Geometry: final body of the model. Coordinates: model frame, mm. Coordinates: 2 decimals unless noted, no trailing zeros. Write each loop counter-clockwise with the first axis right and the second up, starting at its lowest first coordinate (ties: lowest second). Pieces come first, ordered by that corner, then holes. Notation, with made-up numbers: (62.5, 40.25) -> (117.5, 40.25) arc R27 cw to (117.5, 76.25) -> close; hole circle Ø4 at (35, -24.5). An arc over 180 degrees is marked (long way). One line per item, written item: value.
```python
from build123d import *

# Parameters (mm, degrees)
SKETCH1_R           = 25
SKETCH1_R_2         = 9
SKETCH1_R_3         = 2.1
BOSS_EXTRUDE1_DEPTH = 4


with BuildPart() as part:
    # Sketch1 → Boss-Extrude1 (new body)
    with BuildSketch(Plane.XY):
        Circle(SKETCH1_R)
        Circle(SKETCH1_R_2, mode=Mode.SUBTRACT)
        with Locations((0, 20)):
            Circle(SKETCH1_R_3, mode=Mode.SUBTRACT)
        with Locations((-20, 0)):
            Circle(SKETCH1_R_3, mode=Mode.SUBTRACT)
        with Locations((20, 0)):
            Circle(SKETCH1_R_3, mode=Mode.SUBTRACT)
        with Locations((0, -20)):
            Circle(SKETCH1_R_3, mode=Mode.SUBTRACT)
    extrude(amount=BOSS_EXTRUDE1_DEPTH)


solid = part.part
```
(1) Section D-D (z = 1.4). Return the cut outline in (x, y), then the cut area to 3 significant figures.
Responses:
outline: circle Ø50 at (0, 0); hole circle Ø4.2 at (-20, 0); hole circle Ø18 at (0, 0); hole circle Ø4.2 at (0, -20); hole circle Ø4.2 at (0, 20); hole circle Ø4.2 at (20, 0)
area: 1,650 mm2
(2) Section A-A (y = 0). Return the cut outline in (x, z), then the cut area to 3 significant figures.
Responses:
outline: (-25, 0) -> (-22.1, 0) -> (-22.1, 4) -> (-25, 4) -> close; (-17.9, 0) -> (-9, 0) -> (-9, 4) -> (-17.9, 4) -> close; (9, 0) -> (17.9, 0) -> (17.9, 4) -> (9, 4) -> close; (22.1, 0) -> (25, 0) -> (25, 4) -> (22.1, 4) -> close
area: 94.4 mm2
(3) Line query: line 1 (X direction, y = 19.5, z = 0.7); line 2 (Y direction, x = -20, z = 2.6); line 3 (Y direction, x = -19, z = 0.5). Output: solid intervals per line, ascending. Write a range as [from, to].
Responses:
line 1: x = [-15.64, -2.04], [2.04, 15.64]
line 2: y = [-15, -2.1], [2.1, 15]
line 3: y = [-16.25, -1.85], [1.85, 16.25]
(4) Pull-direction query (X, two-part tool) for faces 1 (the flat face through (0, -11, 4)), 2 (the cylindrical face through (23.846, 7.509, 1.972)), 3 (the cylindrical face through (-1.172, 8.923, 1.972)); classes: released by +X, released by -X, zero draft, split by the parting line, or undercut.
Responses:
face 1: zero draft
face 2: split by the parting line
face 3: undercut
(5) First-contact query: pin 1 (14.5 mm diameter, centred on x = 0, y = 0, fed in from +Z); pin 2 (1 mm diameter, centred on x = 4, y = 12, fed in from -Z). Flat tips, straight axial feed; report the tip coordinate or a pass-through.
Responses:
pin 1: passes through
pin 2: stops at z = 0
(6) Section B-B (x = 20). Return the cut outline in (y, z).
Responses:
outline: (-15, 0) -> (-2.1, 0) -> (-2.1, 4) -> (-15, 4) -> close; (2.1, 0) -> (15, 0) -> (15, 4) -> (2.1, 4) -> close
